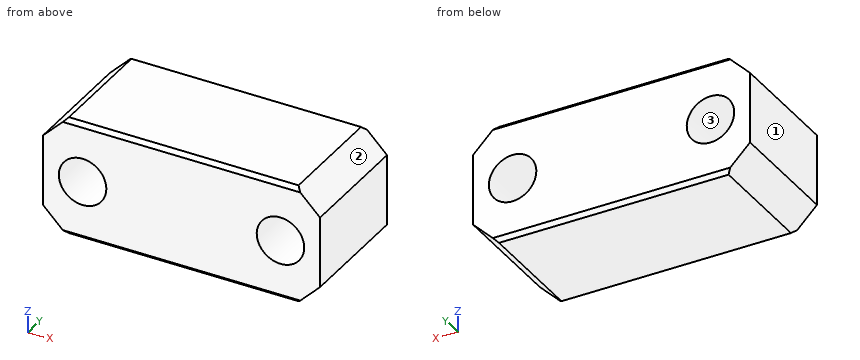
from build123d import *

# Parameters (mm, degrees)
SKETCH1_W           = 35
SKETCH1_H           = 15
BOSS_EXTRUDE1_DEPTH = 15
SKETCH2_R           = 3
CUT_EXTRUDE1_DEPTH  = 15.7
CHAMFER1_SIZE       = 3
CHAMFER2_SIZE       = 0.5


with BuildPart() as part:
    # Sketch1 → Boss-Extrude1 (new body)
    with BuildSketch(Plane(origin=(0, 0, 0), x_dir=(1, 0, 0), z_dir=(0, 1, 0))):
        with Locations((-67.573325782, 9.634846385)):
            Rectangle(SKETCH1_W, SKETCH1_H)
    extrude(amount=BOSS_EXTRUDE1_DEPTH)

    # Sketch2 → Cut-Extrude1 (cut)
    with BuildSketch(Plane(origin=(0, 15, 0), x_dir=(1, 0, 0), z_dir=(0, 1, 0))):
        with Locations(Location((-80.073325782, 9.634846385, 0), (0, 0, 270))):
            Circle(SKETCH2_R)
        with Locations(Location((-55.073325782, 9.634846385, 0), (0, 0, 270))):
            Circle(SKETCH2_R)
    extrude(amount=-CUT_EXTRUDE1_DEPTH, mode=Mode.SUBTRACT)

    # Chamfer1
    chamfer1_edges = [part.edges().sort_by_distance(p)[0] for p in [
        (-85.073325782, 7.5, -17.134846385),
        (-50.073325782, 7.5, -17.134846385),
        (-50.073325782, 7.5, -2.134846385),
        (-85.073325782, 7.5, -2.134846385),
    ]]
    chamfer(chamfer1_edges, length=CHAMFER1_SIZE)

    # Chamfer2
    chamfer2_edges = [part.edges().sort_by_distance(p)[0] for p in [
        (-67.573325782, 0, -17.134846385),
        (-67.573325782, 0, -2.134846385),
        (-67.573325782, 15, -2.134846385),
        (-67.573325782, 15, -17.134846385),
    ]]
    chamfer(chamfer2_edges, length=CHAMFER2_SIZE)


solid = part.part
Source: CAD feature listing. Evaluate the final solid. Frame: model axes, mm. Face numbers are marked on the shaded views. Round coordinates to 2 decimals unless told otherwise and drop trailing zeros. Write each loop counter-clockwise with the first axis right and the second up, starting at its lowest first coordinate (ties: lowest second). Pieces come first, ordered by that corner, then holes. Notation, with made-up numbers: (65, 10.5) - (92, 10.5) arc R23 ccw to (92, 39.5) - close; hole circle Ø10 at (46, -26.5). An arc over 180 degrees is marked (long way). Use CSV: the item, a comma, the result in double quotes. Start each with the question number.
(1) Cut plane D-D, the plane z = -9.25. Return loops of the section in (x, y).
(2) Cut plane B-B, the plane x = -56. Return loops of the section in (y, z), and give its area (3 significant figures).
(3) Material intervals for probe 1 along X at (y, z) = (4, -7); probe 2 along X at (y, z) = (7, -11.5); probe 3 along Z at (x, y) = (-78, 1.5), sorted ascending. Write a range as [from, to].
(4) Mould query, pull axis X, two halves, no side actions, for the marked faces 1, 2 and 3. Classes: pulls with the +X half, pulls with the -X half, needs draft (parallel to the pull), parting line crosses it, or undercut.
(5) Cut plane C-C, the plane y = 3.25. Return loops of the section in (x, z).
(6) Cut plane A-A, the plane z = -7. Return loops of the section in (x, y).
Geometry says:
1,outline,"(-85.07, 0) - (-83.05, 0) - (-83.05, 15) - (-85.07, 15) - close; (-77.1, 0) - (-58.05, 0) - (-58.05, 15) - (-77.1, 15) - close; (-52.1, 0) - (-50.07, 0) - (-50.07, 15) - (-52.1, 15) - close"
2,outline,"(0, -16.63) - (0.5, -17.13) - (14.5, -17.13) - (15, -16.63) - (15, -12.49) - (0, -12.49) - close; (0, -6.78) - (15, -6.78) - (15, -2.63) - (14.5, -2.13) - (0.5, -2.13) - (0, -2.63) - close"
2,area,"139 mm²"
3,probe 1,"[-85.07, -81.51], [-78.64, -56.51], [-53.64, -50.07]"
3,probe 2,"[-85.07, -82.42], [-77.72, -57.42], [-52.72, -50.07]"
3,probe 3,"[-17.13, -11.8], [-7.47, -2.13]"
4,face 1,"pulls with the -X half"
4,face 2,"pulls with the +X half"
4,face 3,"undercut"
5,outline,"(-85.07, -14.13) - (-82.07, -17.13) - (-53.07, -17.13) - (-50.07, -14.13) - (-50.07, -5.13) - (-53.07, -2.13) - (-82.07, -2.13) - (-85.07, -5.13) - close; hole circle Ø6 at (-80.07, -9.63); hole circle Ø6 at (-55.07, -9.63)"
6,outline,"(-85.07, 0) - (-81.51, 0) - (-81.51, 15) - (-85.07, 15) - close; (-78.64, 0) - (-56.51, 0) - (-56.51, 15) - (-78.64, 15) - close; (-53.64, 0) - (-50.07, 0) - (-50.07, 15) - (-53.64, 15) - close"
